Verification items for the finished model (mm, model axes). A direction names the side the tool comes from. Round coordinates to 2 decimals unless told otherwise and drop trailing zeros. Write each loop counter-clockwise with the first axis right and the second up, starting at its lowest first coordinate (ties: lowest second). Pieces come first, ordered by that corner, then holes. Notation, with made-up numbers: (52, -18) -> (65, -18) arc R7 cw to (65, -9) -> close; hole circle Ø5 at (74, -24). An arc over 180 degrees is marked (long way). Use CSV: the item, a comma, the result in double quotes.
```python
from build123d import *

# Parameters (mm, degrees)
SKETCH_1_W                = 140
SKETCH_1_H                = 250
EXTRUDE_1_DEPTH           = 12
HOLE_WIZARD_1_D           = 5.5
HOLE_WIZARD_1_DEPTH       = 15
HOLE_WIZARD_1_CBORE_D     = 10
HOLE_WIZARD_1_CBORE_DEPTH = 5.7
HOLE_WIZARD_1_TIP         = 1.652366702
HOLE_WIZARD_2_D           = 6.6
HOLE_WIZARD_2_DEPTH       = 15
HOLE_WIZARD_2_CBORE_D     = 11
HOLE_WIZARD_2_CBORE_DEPTH = 6.8
HOLE_WIZARD_2_TIP         = 1.982840043
HOLE_WIZARD_3_D           = 5.5
HOLE_WIZARD_3_DEPTH       = 14.4
HOLE_WIZARD_3_CBORE_D     = 10
HOLE_WIZARD_3_CBORE_DEPTH = 5.7
HOLE_WIZARD_3_TIP         = 1.652366702
SKETCH_8_W                = 140
SKETCH_8_H                = 81
CUT_EXTRUDE_1_DEPTH       = 2
HOLE_WIZARD_0_D           = 5.5
HOLE_WIZARD_0_CBORE_D     = 10
HOLE_WIZARD_0_CBORE_DEPTH = 7
HOLE_WIZARD_M5_1_D        = 4.2
FILLET_1_R                = 5


with BuildPart() as part:
    # 草图1 → 凸台-拉伸1 (new body)
    with BuildSketch(Plane.XY):
        Rectangle(SKETCH_1_W, SKETCH_1_H)
    extrude(amount=EXTRUDE_1_DEPTH)

    # 打孔尺寸(%根据)内六角圆柱头螺钉的类型1
    with Locations(Plane.XY.offset(12)):
        with Locations((-18, 112.800000705), (-18, 80.800000705), (18, 80.800000705), (18, 112.800000705)):
            CounterBoreHole(HOLE_WIZARD_1_D / 2, HOLE_WIZARD_1_CBORE_D / 2, HOLE_WIZARD_1_CBORE_DEPTH, depth=HOLE_WIZARD_1_DEPTH)
            with Locations((0, 0, -(HOLE_WIZARD_1_DEPTH + HOLE_WIZARD_1_TIP / 2))):  # 118° drill point
                Cone(0, HOLE_WIZARD_1_D / 2, HOLE_WIZARD_1_TIP, mode=Mode.SUBTRACT)

    # 打孔尺寸(%根据)内六角圆柱头螺钉的类型2
    with Locations(Plane.XY.offset(12)):
        with Locations((37.5, -106.499999647), (-37.5, -106.499999647), (-37.5, -41.499999647), (37.5, -41.499999647)):
            CounterBoreHole(HOLE_WIZARD_2_D / 2, HOLE_WIZARD_2_CBORE_D / 2, HOLE_WIZARD_2_CBORE_DEPTH, depth=HOLE_WIZARD_2_DEPTH)
            with Locations((0, 0, -(HOLE_WIZARD_2_DEPTH + HOLE_WIZARD_2_TIP / 2))):  # 118° drill point
                Cone(0, HOLE_WIZARD_2_D / 2, HOLE_WIZARD_2_TIP, mode=Mode.SUBTRACT)

    # 打孔尺寸(%根据)内六角圆柱头螺钉的类型3
    with Locations(Plane(origin=(0, 0, 0), x_dir=(-1, 0, 0), z_dir=(0, 0, -1))):
        with Locations((0, -105), (0, -55)):
            CounterBoreHole(HOLE_WIZARD_3_D / 2, HOLE_WIZARD_3_CBORE_D / 2, HOLE_WIZARD_3_CBORE_DEPTH, depth=HOLE_WIZARD_3_DEPTH)
            with Locations((0, 0, -(HOLE_WIZARD_3_DEPTH + HOLE_WIZARD_3_TIP / 2))):  # 118° drill point
                Cone(0, HOLE_WIZARD_3_D / 2, HOLE_WIZARD_3_TIP, mode=Mode.SUBTRACT)

    # 草图8 → 切除-拉伸1 (cut)
    with BuildSketch(Plane(origin=(0, 0, 0), x_dir=(-1, 0, 0), z_dir=(0, 0, -1))):
        with Locations((0, -73.999999647)):
            Rectangle(SKETCH_8_W, SKETCH_8_H)
    extrude(amount=-CUT_EXTRUDE_1_DEPTH, mode=Mode.SUBTRACT)

    # 打孔尺寸(%根据)内六角圆柱头螺钉的类型0 (through all)
    with Locations(Plane(origin=(0, 0, 0), x_dir=(-1, 0, 0), z_dir=(0, 0, -1))):
        with Locations((-50, -30), (50, -30)):
            CounterBoreHole(HOLE_WIZARD_0_D / 2, HOLE_WIZARD_0_CBORE_D / 2, HOLE_WIZARD_0_CBORE_DEPTH)

    # M5 螺纹孔1 (through all)
    with Locations(Plane.XY.offset(12)):
        with Locations((30, -95), (60, -95)):
            Hole(HOLE_WIZARD_M5_1_D / 2)

    # 圆角1
    fillet_1_edges = [part.edges().sort_by_distance(p)[0] for p in [
        (-70, 125, 6),
        (70, 125, 6),
        (70, -125, 6),
        (-70, -125, 6),
    ]]
    fillet(fillet_1_edges, radius=FILLET_1_R)


solid = part.part
```
Q1. Section check B-B (x = 37.5). Record the cut outline in (y, z).
Filled in:
outline,"(-125, 0) -> (-114.5, 0) -> (-114.5, 2) -> (-109.8, 2) -> (-109.8, 5.2) -> (-112, 5.2) -> (-112, 12) -> (-125, 12) -> close; (-103.2, 2) -> (-44.8, 2) -> (-44.8, 5.2) -> (-47, 5.2) -> (-47, 12) -> (-101, 12) -> (-101, 5.2) -> (-103.2, 5.2) -> close; (-38.2, 2) -> (-33.5, 2) -> (-33.5, 0) -> (125, 0) -> (125, 12) -> (-36, 12) -> (-36, 5.2) -> (-38.2, 5.2) -> close"
Q2. Section check A-A (y = 112.8). Record the cut outline in (x, z).
Filled in:
outline,"(-70, 0) -> (-20.75, 0) -> (-20.75, 6.3) -> (-23, 6.3) -> (-23, 12) -> (-70, 12) -> close; (-15.25, 0) -> (15.25, 0) -> (15.25, 6.3) -> (13, 6.3) -> (13, 12) -> (-13, 12) -> (-13, 6.3) -> (-15.25, 6.3) -> close; (20.75, 0) -> (70, 0) -> (70, 12) -> (23, 12) -> (23, 6.3) -> (20.75, 6.3) -> close"
Q3. Section check C-C (y = -55). Record the cut outline in (x, z).
Filled in:
outline,"(-70, 2) -> (-5, 2) -> (-5, 5.7) -> (-2.75, 5.7) -> (-2.75, 12) -> (-70, 12) -> close; (2.75, 5.7) -> (5, 5.7) -> (5, 2) -> (70, 2) -> (70, 12) -> (2.75, 12) -> close"
Q4. Mould release check, pull along X, two halves, no side actions. Record for faces 1 (the cylindrical face through (68, 124, 6)), 2 (the flat face through (-1, -125, 6)), 3 (the cylindrical face through (-0.358, -52.273, 8.894)), 4 (the flat face through (47.8, -32.2, 7)): released by +X, released by -X, zero draft, split by the parting line, or undercut.
Filled in:
face 1,"released by +X"
face 2,"zero draft"
face 3,"undercut"
face 4,"undercut"
Q5. Go/stop test with flat-tipped pins: P1, Ø3.5, axis at x = 0, y = -55, coming from the -Z side; P2, Ø5, axis at x = -50.5, y = -29.5, coming from the -Z side; P3, Ø10, axis at x = 33.5, y = -81, coming from the -Z side; P4, Ø3, axis at x = -19, y = 112, coming from the +Z side. Record where each tip stops, or that it passes through.
Filled in:
P1,"through"
P2,"z = 7"
P3,"z = 2"
P4,"z = 6.3"
Q6. Section check D-D (x = -50). Record the cut outline in (y, z), plus the area to 3 significant figures.
Filled in:
outline,"(-125, 0) -> (-114.5, 0) -> (-114.5, 2) -> (-35, 2) -> (-35, 7) -> (-32.75, 7) -> (-32.75, 12) -> (-125, 12) -> close; (-27.25, 7) -> (-25, 7) -> (-25, 0) -> (125, 0) -> (125, 12) -> (-27.25, 12) -> close"
area,"2,740 mm²"
Q7. Material ranges on L1, parallel to X at y = -30.5, z = 3; L2, parallel to Y at x = -37.5, z = 10; L3, parallel to Y at x = -38, z = 4.5, recorded low to high.
Filled in:
L1,"-70 to -54.97, -45.03 to 45.03, 54.97 to 70"
L2,"-125 to -112, -101 to -47, -36 to 125"
L3,"-125 to -109.76, -103.24 to -44.76, -38.24 to 125"
Q8. Access from +Z, -Z, +X, -X, +Y, -Y to the whole of each face (thin tool, end or side, straight path). Record for faces 5 (the cylindrical face through (-17.404, 78.115, 3.106)), 6 (the flat face through (-2.2, -57.2, 5.7)), 7 (the cylindrical face through (33.1, -44.8, 8.6)).
Filled in:
face 5,"+Z, -Z"
face 6,"-Z"
face 7,"+Z"
